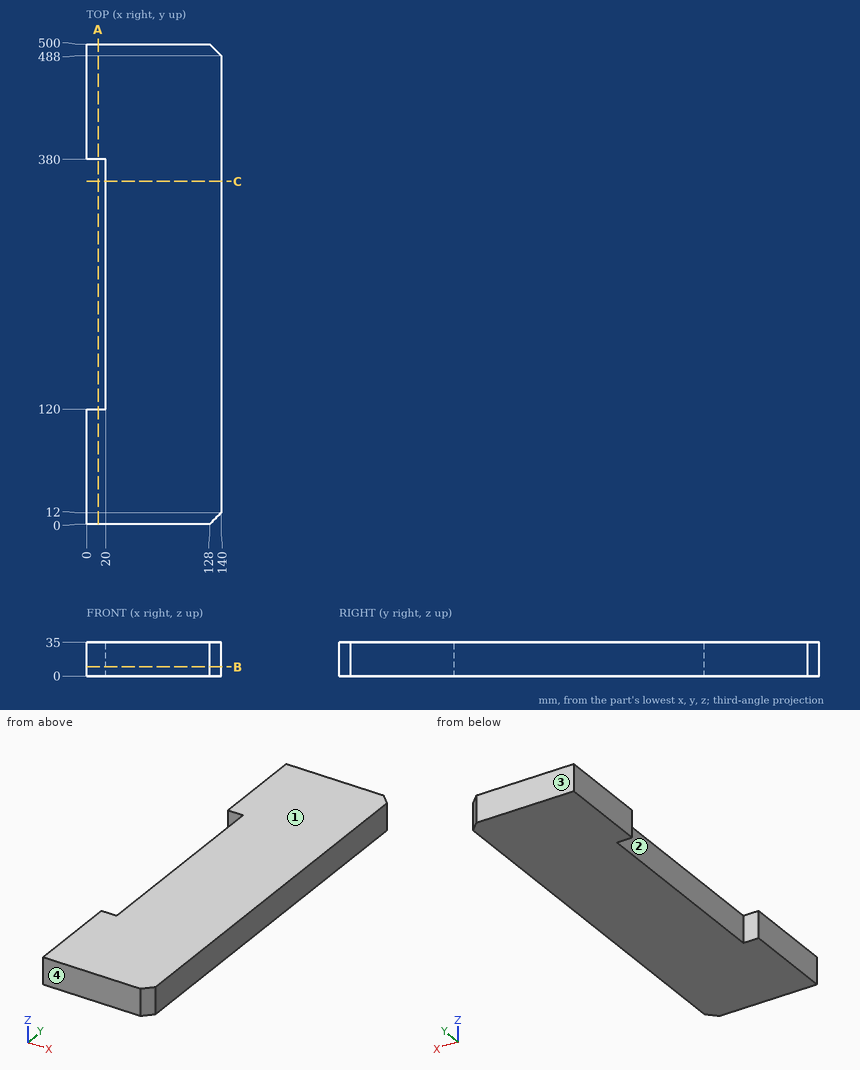
Geometry check sheet. Reference: drawing and pictorial views, mm from the part's lowest x, y, z. Give positions to 0.01 mm unless a question says otherwise; leave off trailing zeros. Order: outer loops, then holes, each group sorted by start corner. A loop starts at its lowest first (then second) coordinate and runs counter-clockwise, first axis right, second up. Notation, with made-up numbers: (14, 36) - (62, 36) arc R21 cw to (62, 53) - close; hole circle Ø5 at (73, 12.5). An arc over 180 degrees is marked (long way). Use one line per item in the form item = value.
1) Depth check by flat-ended pin: pin 1 Ø8 at (y, z) = (184.5, 28.5) entering from -X. Enter the tip coordinate at first touch or a pass-through.
Working result:
pin_1 = 20
2) Material ranges on probe 1 along Y at (x, z) = (15.5, 16); probe 2 along X at (y, z) = (157, 32.5); probe 3 along Y at (x, z) = (130, 31), recorded low to high. Write a range as from..to.
Working result:
probe_1 = 0..120, 380..500
probe_2 = 20..140
probe_3 = 2..498
3) Draft check along Y on the marked faces 1, 2, 3 and 4. Enter one of: released by +Y, released by -Y, zero draft, split by the parting line, or undercut.
Working result:
face_1 = zero draft
face_2 = undercut
face_3 = released by +Y
face_4 = released by -Y
4) Sectioned sample at A-A (x = 12). Record the boundary of the cut face in (y, z), and give its area (3 significant figures).
Working result:
outline = (0, 0) - (120, 0) - (120, 35) - (0, 35) - close; (380, 0) - (500, 0) - (500, 35) - (380, 35) - close
area = 8,400 mm^2
5) Sectioned sample at B-B (z = 9.5). Record the boundary of the cut face in (x, y).
Working result:
outline = (0, 0) - (128, 0) - (140, 12) - (140, 488) - (128, 500) - (0, 500) - (0, 380) - (20, 380) - (20, 120) - (0, 120) - close
6) Sectioned sample at C-C (y = 357). Record the boundary of the cut face in (x, z).
Working result:
outline = (20, 0) - (140, 0) - (140, 35) - (20, 35) - close
